Source: CAD feature listing. Evaluate the final solid. Frame: model axes, mm. Give positions to 0.01 mm unless a question says otherwise; leave off trailing zeros. Write each loop counter-clockwise with the first axis right and the second up, starting at its lowest first coordinate (ties: lowest second). Pieces come first, ordered by that corner, then holes.
```python
from build123d import *

# Parameters (mm, degrees)
SKETCH_1_R             = 8.5
EXTRUDE_1_DEPTH        = 35
HOLE_WIZARD_M6_1_D     = 5
HOLE_WIZARD_M6_1_DEPTH = 15
HOLE_WIZARD_M6_1_TIP   = 1.502151548
CHAMFER_1_SIZE         = 0.5
SKETCH_4_W             = 1.1
SKETCH_4_H             = 2.765489895


with BuildPart() as part:
    # 草图1 → 凸台-拉伸1 (new body)
    with BuildSketch(Plane(origin=(0, 0, 0), x_dir=(0, 0, -1), z_dir=(1, 0, 0))):
        Circle(SKETCH_1_R)
    extrude(amount=EXTRUDE_1_DEPTH)

    # M6 螺纹孔1
    with Locations(Plane.ZY):
        with Locations((0, 0)):
            Hole(HOLE_WIZARD_M6_1_D / 2, depth=HOLE_WIZARD_M6_1_DEPTH)
            with Locations((0, 0, -(HOLE_WIZARD_M6_1_DEPTH + HOLE_WIZARD_M6_1_TIP / 2))):  # 118° drill point
                Cone(0, HOLE_WIZARD_M6_1_D / 2, HOLE_WIZARD_M6_1_TIP, mode=Mode.SUBTRACT)

    # 倒角1
    chamfer_1_edges = [part.edges().sort_by_distance(p)[0] for p in [
        (0, 0, 8.5),
        (35, 0, 8.5),
    ]]
    chamfer(chamfer_1_edges, length=CHAMFER_1_SIZE)

    # 草图4 → 切除-旋转1 (revolve, cut)
    with BuildSketch(Plane(origin=(0, 0, 0), x_dir=(1, 0, 0), z_dir=(0, 1, 0)), mode=Mode.PRIVATE) as cut_revolve_1_sk:
        with Locations((32.55, 9.482744948)):
            Rectangle(SKETCH_4_W, SKETCH_4_H)
    revolve(cut_revolve_1_sk.sketch.rotate(Axis((-5.277682127, 0, 0), (1, 0, 0)), 180), axis=Axis((-5.277682127, 0, 0), (1, 0, 0)), mode=Mode.SUBTRACT)


solid = part.part
```
1. Section query B-B (x = 18.5). Return loops of the section in (y, z).
2. Pull-direction query (X, two-part tool) for faces 1 (the cylindrical face through (7.6, -2.44, 0.54)), 2 (the cylindrical face through (32.6, -6.8, 4.4)), 3 (the flat face through (35, 0, 0)), 4 (the conical face through (16.241, -0.424, -0.094)); classes: pulls with the +X half, pulls with the -X half, needs draft (parallel to the pull), parting line crosses it, or undercut.
3. Section query A-A (x = 13.5). Return loops of the section in (y, z), plus the area to 3 significant figures.
4. Pin query (flat end, axial travel): P1, Ø6, axis at x = 16, y = 5, coming from the -Z side; P2, Ø5, axis at x = 18.5, z = 5.5, coming from the +Y side; P3, Ø4, axis at x = 13, z = -2.5, coming from the -Y side. Return the tip coordinate at first contact, or that it passes through.
5. Line query: probe 1 along Z at (x, y) = (7.25, 0); probe 2 along Z at (x, y) = (1, 2.25). Output: solid intervals per line, ascending.
The answers:
1. outline: circle Ø17 at (0, 0)
2. face 1: needs draft
2. face 2: undercut
2. face 3: pulls with the +X half
2. face 4: pulls with the -X half
3. outline: circle Ø17 at (0, 0); hole circle Ø5 at (0, 0)
3. area: 207 mm2
4. P1: stops at z = -8.26
4. P2: stops at y = 7.95
4. P3: stops at y = -8.49
5. probe 1: z = -8.5 to -2.5, 2.5 to 8.5
5. probe 2: z = -8.2 to -1.09, 1.09 to 8.2
